from build123d import *


with BuildPart() as part:
    # Sketch2 → Revolve1 (revolve)
    with BuildSketch(Plane.XY):
        Polygon((50, 0), (55, 0), (55, 6), (54, 6), (51.5, 8), (51, 8), (50, 6), align=None)
    revolve(axis=Axis((0, -1000, 0), (0, 1, 0)))


solid = part.part
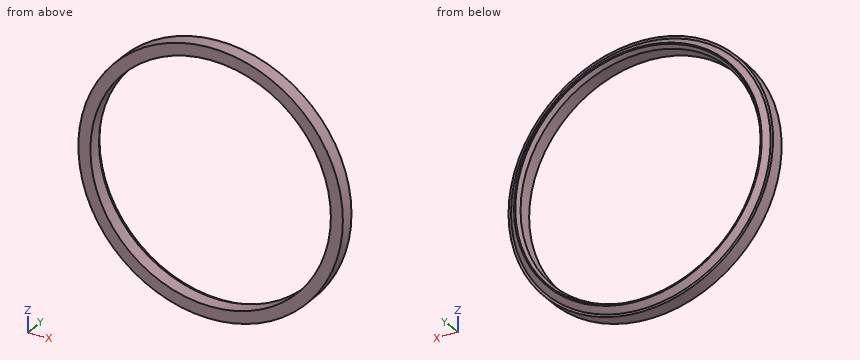
Here's how the part is built. I have some questions about the finished solid (model axes, mm). Round coordinates to 2 decimals unless told otherwise and drop trailing zeros. Write each loop counter-clockwise with the first axis right and the second up, starting at its lowest first coordinate (ties: lowest second). Pieces come first, ordered by that corner, then holes.
1. Suppose I cut it at B-B (x = 0). List the corners of the cut face in (y, z) for me.
2. Suppose I cut it at A-A (z = 0). List the corners of the cut face in (x, y) for me.
3. Will these pins go through, and if not, where does the flat tip stop? pin 1 Ø1 at (y, z) = (6, -6.5) entering from -X; pin 2 Ø2 at (y, z) = (2.5, 2) entering from +X; pin 3 Ø2 at (y, z) = (3.5, -33.5) entering from +X.
4. Suppose I cut it at C-C (y = 1.25). List the corners of the cut face in (x, z) for me.
5. I need wall thicknesses on L1, parallel to X at y = 2, z = 0; L2, parallel to Z at x = 45, y = 5.25. Which ranges of each line are inside material? Lowest first, please.
Answer sheet:
1. outline: (0, -55) - (6, -55) - (6, -54) - (8, -51.5) - (8, -51) - (6, -50) - (0, -50) - close; (0, 50) - (6, 50) - (8, 51) - (8, 51.5) - (6, 54) - (6, 55) - (0, 55) - close
2. outline: (-55, 0) - (-50, 0) - (-50, 6) - (-51, 8) - (-51.5, 8) - (-54, 6) - (-55, 6) - close; (50, 0) - (55, 0) - (55, 6) - (54, 6) - (51.5, 8) - (51, 8) - (50, 6) - close
3. pin 1: stops at x = -54.67
3. pin 2: stops at x = 54.99
3. pin 3: stops at x = 44.37
4. outline: circle Ø110 at (0, 0); hole circle Ø100 at (0, 0)
5. L1: x = -55 to -50, 50 to 55
5. L2: z = -31.62 to -21.79, 21.79 to 31.62
